Work out the finished part from the listing and answer in its coordinate system (mm). A direction names the side the tool comes from. Give positions to 0.01 mm unless a question says otherwise; leave off trailing zeros. Loops run counter-clockwise (first coordinate to the right, second up) from the corner with the lowest first, then second, coordinate; pieces in that order, holes last. Notation, with made-up numbers: M 87.25,41.25 L 138.25,41.25 A15 ccw 138.25,50.25 Z; hole C 89.5,-32 d11. An arc over 180 degrees is marked long. Write item = value, one per line. Start each with the question number.
1. Section A-A on y = 0 is taken. Determine the outline of the cut face in (x, z).
2. Section D-D on x = 9 is taken. Determine the outline of the cut face in (y, z), plus the area to 3 significant figures.
3. The mould has two halves that part along X. Classify faces 4 (the face through (9, 0, 75)), 5 (the face through (0, 0, 30)), 6 (the face through (-17.169, 5.407, 14.79)), 7 (the face through (28.284, -4.3, 18.1)): released by +X, released by -X, zero draft, split by the parting line, or undercut.
4. Section C-C on z = 15 is taken. Determine the outline of the cut face in (x, y), plus the area to 3 significant figures.
5. For faces 1 (the face through (28.076, 6.007, 42.465)), 2 (the face through (22.696, 0.224, 9.905)), 3 (the face through (29, 0, 30)), determine the directions among +Z, -Z, +X, -X, +Y, -Y from which every point of the face is accessible in a straight line to the end or side of a thin tool.
6. Consider L1, parallel to Z at x = 20, y = 0; L2, parallel to Z at x = 24.5, y = 0; L3, parallel to X at y = 0, z = 21. Determine where each line is inside the solid, lowest interval first. Write a range as [from, to].
7. Section B-B on x = 21.5 is taken. Determine the outline of the cut face in (y, z).
8. Flat-ended cylindrical pins translate along their axes: pin 1 Ø1 at (x, z) = (10, 43) entering from -Y; pin 2 Ø8 at (y, z) = (0, 15) entering from +X; pin 3 Ø5 at (y, z) = (-2, 56.5) entering from +X. Find the tip coordinate at first contact, or state that the pin passes through.
```python
from build123d import *

# Parameters (mm, degrees)
SKETCH_1_R              = 30
EXTRUDE_1_DEPTH         = 40
SKETCH_2_R              = 20
EXTRUDE_2_DEPTH         = 5
SKETCH_3_R              = 15
EXTRUDE_3_DEPTH         = 30
SKETCH_5_R              = 18
CUT_EXTRUDE_1_DEPTH     = 30
HOLE_WIZARD_M12_1_D     = 10.2
HOLE_WIZARD_M12_1_DEPTH = 29.25
HOLE_WIZARD_M12_1_TIP   = 3.064389157


with BuildPart() as part:
    # 草图1 → 凸台-拉伸1 (new body)
    with BuildSketch(Plane.XY):
        Circle(SKETCH_1_R)
    extrude(amount=EXTRUDE_1_DEPTH)

    # 草图2 → 凸台-拉伸2 (add)
    with BuildSketch(Plane.XY.offset(40)):
        with Locations((9, 0)):
            Circle(SKETCH_2_R)
    extrude(amount=EXTRUDE_2_DEPTH)

    # 草图3 → 凸台-拉伸3 (add)
    with BuildSketch(Plane.XY.offset(45)):
        with Locations((9, 0)):
            Circle(SKETCH_3_R)
    extrude(amount=EXTRUDE_3_DEPTH)

    # 草图5 → 切除-拉伸1 (cut)
    with BuildSketch(Plane(origin=(0, 0, 0), x_dir=(-1, 0, 0), z_dir=(0, 0, -1))):
        Circle(SKETCH_5_R)
        Polygon((-30.259977001, 10), (-28.284271247, 10), (-28.284271247, -10), (-32.220348536, -10), (-32.220348536, 10), align=None)
    extrude(amount=-CUT_EXTRUDE_1_DEPTH, mode=Mode.SUBTRACT)

    # M12 螺纹孔1
    with Locations(Plane(origin=(28.284271247, 0, 0), x_dir=(0, 0, -1), z_dir=(1, 0, 0))):
        with Locations((-15, 0)):
            Hole(HOLE_WIZARD_M12_1_D / 2, depth=HOLE_WIZARD_M12_1_DEPTH)
            with Locations((0, 0, -(HOLE_WIZARD_M12_1_DEPTH + HOLE_WIZARD_M12_1_TIP / 2))):  # 118° drill point
                Cone(0, HOLE_WIZARD_M12_1_D / 2, HOLE_WIZARD_M12_1_TIP, mode=Mode.SUBTRACT)


solid = part.part
```
Verdict:
q1.outline = M -30,0 L -18,0 L -18,30 L 18,30 L 18,20.1 L 28.28,20.1 L 28.28,30 L 30,30 L 30,40 L 29,40 L 29,45 L 24,45 L 24,75 L -6,75 L -6,45 L -11,45 L -11,40 L -30,40 Z; M 18,0 L 28.28,0 L 28.28,9.9 L 18,9.9 Z
q2.outline = M -28.62,0 L -15.59,0 L -15.59,30 L 15.59,30 L 15.59,0 L 28.62,0 L 28.62,40 L 20,40 L 20,45 L 15,45 L 15,75 L -15,75 L -15,45 L -20,45 L -20,40 L -28.62,40 Z
q2.area = 2,450 mm2
q3.face_4 = zero draft
q3.face_5 = undercut
q3.face_6 = undercut
q3.face_7 = released by +X
q4.outline = M 17.26,-5.1 A18 cw long 17.26,5.1 L 28.28,5.1 L 28.28,10 A30 ccw long 28.28,-10 L 28.28,-5.1 Z
q4.area = 1,680 mm2
q5.face_1 = +Z
q5.face_2 = +X
q5.face_3 = -Z, +X, +Y, -Y
q6.L1 = [0, 9.9], [20.1, 75]
q6.L2 = [0, 9.9], [20.1, 45]
q6.L3 = [-30, -18], [18, 28.28]
q7.outline = M -20.92,0 L 20.92,0 L 20.92,40 L 15.61,40 L 15.61,45 L 8.29,45 L 8.29,75 L -8.29,75 L -8.29,45 L -15.61,45 L -15.61,40 L -20.92,40 Z; hole C 0,15 d10.2
q8.pin_1 = -19.99
q8.pin_2 = -17.55
q8.pin_3 = 24
